Part model, mm, in its own coordinate system. Face numbers are marked on the shaded views. A direction names the side the tool comes from. Give positions to 0.01 mm unless a question says otherwise; leave off trailing zeros. Order: outer loops, then holes, each group sorted by start corner. A loop starts at its lowest first (then second) coordinate and runs counter-clockwise, first axis right, second up.
from build123d import *

# Parameters (mm, degrees)
HEAD_CHAMFER_3MM_SIZE      = 3
EDGE_CHAMFER_2MM_SIZE      = 2
HEAD_CROSS_HOLE_DEPTH      = 157.642906
HEAD_CROSS_HOLE_DEPTH_BACK = 157.642906
CROSS_HOLE_SKETCH_R        = 3


with BuildPart() as part:
    # Bolt Profile Sketch → Bolt Body Revolve (revolve)
    with BuildSketch(Plane.XY, mode=Mode.PRIVATE) as bolt_body_revolve_sk:
        Polygon((155, 0), (155, 16), (135, 16), (135, 9), (83.46, 9), (83.46, 7), (81.46, 7), (81.46, 9), (61.46, 9), (61.46, 7), (59.46, 7), (59.46, 9), (0, 9), (0, 0), align=None)
    revolve(bolt_body_revolve_sk.sketch.rotate(Axis((0, 0, 0), (1, 0, 0)), 90), axis=Axis((0, 0, 0), (1, 0, 0)))

    # Head Chamfer 3mm
    head_chamfer_3mm_edges = [part.edges().sort_by_distance(p)[0] for p in [
        (135, 0, -16),
        (155, 0, -16),
    ]]
    chamfer(head_chamfer_3mm_edges, length=HEAD_CHAMFER_3MM_SIZE)

    # Edge Chamfer 2mm
    edge_chamfer_2mm_edges = [part.edges().sort_by_distance(p)[0] for p in [
        (0, 0, -9),
    ]]
    chamfer(edge_chamfer_2mm_edges, length=EDGE_CHAMFER_2MM_SIZE)

    # Cross Hole Sketch → Head Cross Hole (cut, two sides: drawn at the far end of the back side and taken through both)
    with BuildSketch(Plane.XY.offset(-HEAD_CROSS_HOLE_DEPTH_BACK)):
        with Locations((145, 0)):
            Circle(CROSS_HOLE_SKETCH_R)
    extrude(amount=HEAD_CROSS_HOLE_DEPTH + HEAD_CROSS_HOLE_DEPTH_BACK, mode=Mode.SUBTRACT)


solid = part.part
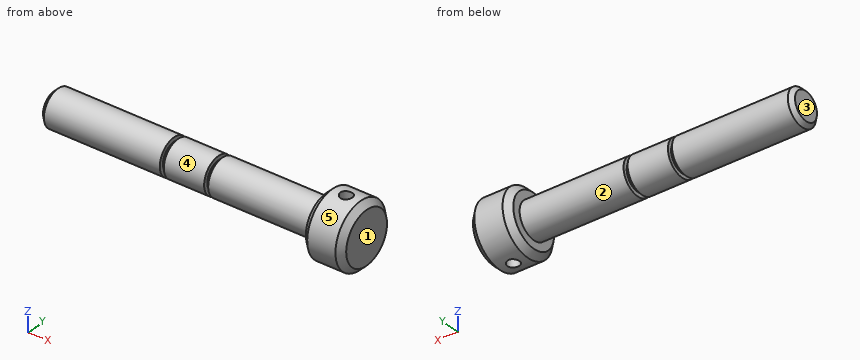
Item 1: Band-saw the part on C-C on x = 21.5. List the corners of the cut face in (y, z), plus the area to 3 significant figures.
Item 2: Drop flat-ended pins along their axis: P1, Ø12, axis at x = 80.5, z = -12.5, coming from the +Y side; P2, Ø3, axis at x = 60.5, z = -2.5, coming from the -Y side; P3, Ø1.5, axis at x = 97.5, z = 6.5, coming from the +Y side; P4, Ø5.5, axis at x = 145, y = 0, coming from the +Z side. Give the stop position or say it passes through.
Item 3: Drill centre lines: probe 1 along X at (y, z) = (0, -4); probe 2 along X at (y, z) = (1.5, 2); probe 3 along Y at (x, z) = (33.5, 0). Where is each one in solid material? Low to high.
Item 4: Which spindle directions (+Z, -Z, +X, -X, +Y, -Y) get a long thin tool onto all of the face, cutting with end or side? Do the marked faces 4 and 5. Say none if no direction does.
Item 5: Band-saw the part on D-D on x = 145. List the corners of the cut face in (y, z), plus the area to 3 significant figures.
Item 6: Pull direction X, two halves, no side cores. Call the marked faces 1, 2 and 3: released by +X, released by -X, zero draft, split by the parting line, or undercut.
Working result:
1. outline: circle Ø18 at (0, 0)
1. area: 254 mm2
2. P1: stops at y = 6.22
2. P2: stops at y = -8.9
2. P3: stops at y = 6.92
2. P4: passes through
3. probe 1: x = 0 to 142, 148 to 155
3. probe 2: x = 0 to 142.4, 147.6 to 155
3. probe 3: y = -9 to 9
4. face 4: -X
4. face 5: +X, -X
5. outline: (-3, -15.72) - (-3, 15.72) arc R16 ccw to start; (3, -15.72) arc R16 ccw to (3, 15.72) - close
5. area: 613 mm2
6. face 1: released by +X
6. face 2: zero draft
6. face 3: released by -X
